Build history of the part. All positions in model axes, mm. A direction names the side the tool comes from. Give positions to 0.01 mm unless a question says otherwise; leave off trailing zeros. Order: outer loops, then holes, each group sorted by start corner. A loop starts at its lowest first (then second) coordinate and runs counter-clockwise, first axis right, second up. Notation, with made-up numbers: (84.25, 8) -> (126.25, 8) arc R17 ccw to (126.25, 26) -> close; hole circle Ø8 at (85, -22). An arc over 180 degrees is marked (long way). One line per item, written item: value. Start each with the question number.
(1) Probe line 1 (X direction, y = 35.5, z = 48); line 2 (Y direction, x = 71.5, z = 55); line 3 (Z direction, x = 32.5, y = 29.5). List the from-to ranges inside material, lowest first.
(2) Two-plate mould, pull along Z, no slides. Class faces 1 (the flat face through (50, 30, 105)), 2 (the flat face through (60, 23, 60)), 3 (the flat face through (100, 30, 10)): +Z half, -Z half, draft (parallel to the pull), parting line (faces both ways), or undercut.
(3) Saw through at A-A on x = 50. Give the cut face in (y, z), plus the area to 3 significant figures.
(4) Which spindle directions (+Z, -Z, +X, -X, +Y, -Y) get a long thin tool onto all of the face, cutting with end or side? Do faces 4 (the flat face through (66, 30, 90)), 5 (the flat face through (93, 30, 20)), 6 (the flat face through (40, 23, 61)), 7 (the flat face through (25, 30, 47)). Say none if no direction does.
(5) Saw through at B-B on y = 39. Give the cut face in (x, z).
(6) Saw through at D-D on y = 30. Count the separate pieces of the cut face and the enclosed holes in it, plus the area to 3 significant figures.
(7) Saw through at C-C on z = 31. Give the cut face in (x, y), plus the area to 3 significant figures.
(8) Pin check, flat tips, straight feed: pin 1 (1 mm diameter, centred on y = 20, z = 58, fed in from -X); pin 2 (20 mm diameter, centred on x = 92.5, y = 24, fed in from +Z); pin 3 (2 mm diameter, centred on y = 53.5, z = 28.5, fed in from +X). Stop position of each tip, or through.
```python
from build123d import *

# Parameters (mm, degrees)
BASE_PLATE_SKETCH_W      = 100
BASE_PLATE_SKETCH_H      = 60
BASE_PLATE_DEPTH         = 20
UPRIGHT_BLOCK_DEPTH      = 60
TOP_SLOT_DEPTH           = 60
NOTCH_SKETCH_R           = 5
NOTCH_CUT_DEPTH          = 20
CROSS_HOLE_A_15_SKETCH_R = 7.5
CROSS_HOLE_A_15_DEPTH    = 25
CROSS_START              = -25
CROSS_HOLE_B_15_SKETCH_R = 7.5
CROSS_HOLE_B_15_DEPTH    = 25
PIN_BOSS_30_SKETCH_R     = 15
PIN_BOSS_30_DEPTH        = 15


with BuildPart() as part:
    # Base Plate Sketch → Base Plate (new body)
    with BuildSketch(Plane.XY):
        with Locations((50, 30)):
            Rectangle(BASE_PLATE_SKETCH_W, BASE_PLATE_SKETCH_H)
    extrude(amount=BASE_PLATE_DEPTH)

    # Upright Block Sketch → Upright Block (add)
    with BuildSketch(Plane.XZ):
        Polygon((50, 20), (25, 20), (25, 90), (75, 90), (75, 20), align=None)
    extrude(amount=-UPRIGHT_BLOCK_DEPTH)

    # Top Slot Sketch → Top Slot (cut)
    with BuildSketch(Plane.XZ):
        with BuildLine():
            Line((40, 76.29728725), (40, 36.29728725))
            ThreePointArc((40, 36.29728725), (50, 26.29728725), (60, 36.29728725))
            Line((60, 36.29728725), (60, 76.29728725))
            ThreePointArc((60, 76.29728725), (50, 86.29728725), (40, 76.29728725))
        make_face()
    extrude(amount=-TOP_SLOT_DEPTH, mode=Mode.SUBTRACT)

    # Notch Sketch → Notch Cut (cut)
    with BuildSketch(Plane.XY.offset(20)):
        with Locations((87.5, 30)):
            Circle(NOTCH_SKETCH_R)
        with Locations((13.016158592, 30)):
            Circle(NOTCH_SKETCH_R)
    extrude(amount=-NOTCH_CUT_DEPTH, mode=Mode.SUBTRACT)

    # Cross Hole A Ø15 Sketch → Cross Hole A Ø15 (cut)
    with BuildSketch(Plane(origin=(75, 0, 0), x_dir=(0, 0, -1), z_dir=(1, 0, 0))):
        with Locations((-55, 30)):
            Circle(CROSS_HOLE_A_15_SKETCH_R)
    extrude(amount=-CROSS_HOLE_A_15_DEPTH, mode=Mode.SUBTRACT)

    # Cross Hole B Ø15 Sketch → Cross Hole B Ø15 (cut)
    with BuildSketch(Plane.ZY.offset(-25).offset(CROSS_START)):
        with Locations(Location((55, 30, 0), (0, 0, 180))):
            Circle(CROSS_HOLE_B_15_SKETCH_R)
    extrude(amount=CROSS_HOLE_B_15_DEPTH, mode=Mode.SUBTRACT)

    # Pin Boss Ø30 Sketch → Pin Boss Ø30 (add)
    with BuildSketch(Plane.XY.offset(90)):
        with Locations((50, 30)):
            Circle(PIN_BOSS_30_SKETCH_R)
    extrude(amount=PIN_BOSS_30_DEPTH)


solid = part.part
```
Results below:
1. line 1: x = 25 to 40, 60 to 75
1. line 2: y = 0 to 22.5, 37.5 to 60
1. line 3: z = 0 to 47.52, 62.48 to 90
2. face 1: +Z half
2. face 2: undercut
2. face 3: draft
3. outline: (0, 0) -> (60, 0) -> (60, 26.3) -> (0, 26.3) -> close; (0, 86.3) -> (60, 86.3) -> (60, 90) -> (45, 90) -> (45, 105) -> (15, 105) -> (15, 90) -> (0, 90) -> close
3. area: 2,250 mm²
4. face 4: +Z
4. face 5: +Z, +X, +Y, -Y
4. face 6: +Y, -Y
4. face 7: +Z, -X, +Y, -Y
5. outline: (0, 0) -> (100, 0) -> (100, 20) -> (75, 20) -> (75, 90) -> (62, 90) -> (62, 105) -> (38, 105) -> (38, 90) -> (25, 90) -> (25, 20) -> (0, 20) -> close; hole (40, 36.3) arc R10 ccw to (60, 36.3) -> (60, 76.3) arc R10 ccw to (40, 76.3) -> close
6. separate pieces: 4
6. enclosed holes: 0
6. area: 3,990 mm²
7. outline: (25, 0) -> (41.52, 0) -> (41.52, 60) -> (25, 60) -> close; (58.48, 0) -> (75, 0) -> (75, 60) -> (58.48, 60) -> close
7. area: 1,980 mm²
8. pin 1: stops at x = 25
8. pin 2: stops at z = 20
8. pin 3: stops at x = 75
